```python
from build123d import *

# Parameters (mm, degrees)
EXTRUDE_1_DEPTH     = 26
FILLET_1_R          = 1
FILLET_2_R          = 3
FILLET_3_R          = 2
SKETCH_2_R          = 3.25
CUT_EXTRUDE_1_DEPTH = 38.215588132
HOLE_WIZARD_M3_1_D  = 2.5


with BuildPart() as part:
    # 草图1 → 拉伸-薄壁1 (new body)
    with BuildSketch(Plane.XY):
        Polygon((0, 0), (20, 0), (20, 15), (22, 15), (22, -2), (0, -2), align=None)
    extrude(amount=EXTRUDE_1_DEPTH)

    # 圆角1
    fillet_1_edges = [part.edges().sort_by_distance(p)[0] for p in [
        (20, 0, 13),
    ]]
    fillet(fillet_1_edges, radius=FILLET_1_R)

    # 圆角2
    fillet_2_edges = [part.edges().sort_by_distance(p)[0] for p in [
        (22, -2, 13),
    ]]
    fillet(fillet_2_edges, radius=FILLET_2_R)

    # 圆角3
    fillet_3_edges = [part.edges().sort_by_distance(p)[0] for p in [
        (0, -1, 26),
        (0, -1, 0),
        (21, 15, 0),
        (21, 15, 26),
    ]]
    fillet(fillet_3_edges, radius=FILLET_3_R)

    # 草图2 → 切除-拉伸1 (cut, through all)
    with BuildSketch(Plane(origin=(0, 0, 0), x_dir=(1, 0, 0), z_dir=(0, 1, 0))):
        with Locations(Location((8, -13, 0), (0, 0, 270))):
            Circle(SKETCH_2_R)
    extrude(amount=-CUT_EXTRUDE_1_DEPTH, mode=Mode.SUBTRACT)

    # M3 螺纹孔1 (through all)
    with Locations(Plane(origin=(22, 0, 0), x_dir=(0, 0, -1), z_dir=(1, 0, 0))):
        with Locations((-22.5, 12), (-3.5, 12)):
            Hole(HOLE_WIZARD_M3_1_D / 2)


solid = part.part
```
Build history of the part. All positions in model axes, mm. A direction names the side the tool comes from. Round coordinates to 2 decimals unless told otherwise and drop trailing zeros. Write each loop counter-clockwise with the first axis right and the second up, starting at its lowest first coordinate (ties: lowest second). Pieces come first, ordered by that corner, then holes.
1) Mould opens along Z. For faces 3 (the cylindrical face through (0.57, -0.99, 25.4)), 4 (the cylindrical face through (20.986, 13.054, 23.172)), 5 (the flat face through (0, -1, 13)) say: +Z half, -Z half, draft (parallel to the pull), parting line (faces both ways), or undercut.
2) Band-saw the part on C-C, the plane x = 8. List the corners of the cut face in (y, z), and give its area (3 significant figures).
3) Drill centre lines: probe 1 along Y at (x, z) = (4.5, 23.75); probe 2 along Y at (x, z) = (20.8, 22.5); probe 3 along X at (y, z) = (9.5, 19). Where is each one in solid material? Low to high.
4) 3-axis set-ups, long thin cutter, end or side, ignore diameter. For faces 1 (the cylindrical face through (21.01, 14.4, 0.57)), 2 (the flat face through (20, 8, 13)): which of +Z, -Z, +X, -X, +Y, -Y reach the whole face in a straight line?
5) Band-saw the part on A-A, the plane z = 3.5. List the corners of the cut face in (x, y).
6) Band-saw the part on B-B, the plane y = 12. List the corners of the cut face in (x, z).
7) Pin check, flat tips, straight feed: pin 1 (5 mm diameter, centred on x = 13, z = 13.5, fed in from +Y); pin 2 (3 mm diameter, centred on y = 12, z = 3.5, fed in from -X); pin 3 (10.5 mm diameter, centred on x = 8, z = 13, fed in from -Y). Stop position of each tip, or through.
8) Band-saw the part on D-D, the plane z = 13. List the corners of the cut face in (x, y), and give its area (3 significant figures).
Ans:
1. face 3: +Z half
1. face 4: undercut
1. face 5: draft
2. outline: (-2, 0) - (0, 0) - (0, 9.75) - (-2, 9.75) - close; (-2, 16.25) - (0, 16.25) - (0, 26) - (-2, 26) - close
2. area: 39.0 mm2
3. probe 1: y = -2 to 0
3. probe 2: y = -1.4 to 10.75, 13.25 to 15
3. probe 3: x = 20 to 22
4. face 1: -Z, +X, -X, +Y
4. face 2: +Z, -Z, -X, +Y
5. outline: (0, -2) - (19, -2) arc R3 ccw to (22, 1) - (22, 10.75) - (20, 10.75) - (20, 1) arc R1 cw to (19, 0) - (0, 0) - close; (20, 13.25) - (22, 13.25) - (22, 15) - (20, 15) - close
6. outline: (20, 0) - (22, 0) - (22, 2.25) - (20, 2.25) - close; (20, 4.75) - (22, 4.75) - (22, 21.25) - (20, 21.25) - close; (20, 23.75) - (22, 23.75) - (22, 26) - (20, 26) - close
7. pin 1: stops at y = 0
7. pin 2: stops at x = 20
7. pin 3: stops at y = -2
8. outline: (0, -2) - (4.75, -2) - (4.75, 0) - (0, 0) - close; (11.25, -2) - (19, -2) arc R3 ccw to (22, 1) - (22, 15) - (20, 15) - (20, 1) arc R1 cw to (19, 0) - (11.25, 0) - close
8. area: 59.3 mm2
